Could you check a few things on this model? Use its own coordinates, in mm. Coordinates: 2 decimals unless noted, no trailing zeros. Use a Markdown table: item, result. Add a question column.
1) Will these pins go through, and if not, where does the flat tip stop? pin 1 Ø6 at (x, y) = (-6.5, -4) entering from +Z; pin 2 Ø1 at (x, z) = (-10, 6.5) entering from -Y; pin 3 Ø5 at (x, z) = (14.5, 5.5) entering from +Y; pin 4 Ø3 at (y, z) = (3.5, 1) entering from -X.
2) If we section it at A-A (y = 12.5): Give the number of separate pieces and of enclosed holes in the cut face, plus the area to 3 significant figures.
3) If I drill on L1, parallel to Y at x = -11, z = 4.5; L2, parallel to X at y = -10.5, z = 4.25; L3, parallel to Y at x = -11, z = 1.5, over which ranges is the centre line in solid material (lowest first)? Write a range as [from, to].
```python
from build123d import *

# Parameters (mm, degrees)
BASE_EXTRUDE_DEPTH      = 0.001
BASE_EXTRUDE_DEPTH_BACK = 0.001
SKETCH6_W               = 6.42
SKETCH6_H               = 6.76
SKETCH8_R               = 20.30887065
SKETCH8_R_2             = 13.5
BOSS_EXTRUDE1_DEPTH     = 6.46
CUT_EXTRUDE1_DEPTH      = 31.552378082
CUT_EXTRUDE1_DEPTH_BACK = 31.552378082


with BuildPart() as part:
    # Sketch6 → Base-Extrude (new, two sides: drawn at the far end of the back side and taken through both)
    with BuildSketch(Plane(origin=(-9.545941546, 9.545941546, 7.14), x_dir=(0.05931115895295759, 0.059311158952956106, -0.996475977054798), z_dir=(0.7046149206649441, 0.7046149206649323, 0.08387864539133799)).offset(-BASE_EXTRUDE_DEPTH_BACK)):
        with Locations((3.23, 3.4)):
            Rectangle(SKETCH6_W, SKETCH6_H)
    extrude(amount=BASE_EXTRUDE_DEPTH + BASE_EXTRUDE_DEPTH_BACK)

    # Sketch8 → Boss-Extrude1 (add)
    with BuildSketch(Plane(origin=(-0.420803093, -0.420803093, 7.069836103), x_dir=(0.9982394983905275, -0.0038244762114057976, 0.05918848903914046), z_dir=(-0.05931115895295754, -0.05931115895295616, 0.996475977054798))):
        with Locations(Location((0, 0, 0), (0, 0, 0.219513325))):
            Circle(SKETCH8_R)
        with Locations(Location((0, 0, 0), (0, 0, 0.219513325))):
            Circle(SKETCH8_R_2, mode=Mode.SUBTRACT)
    extrude(amount=-BOSS_EXTRUDE1_DEPTH)

    # Sketch9 → Cut-Extrude1 (cut, two sides: drawn at the far end of the back side and taken through both)
    with BuildSketch(Plane.XY.offset(-CUT_EXTRUDE1_DEPTH_BACK)):
        Polygon((-34.048869909, 36.453032965), (0.95291576, 1.451247296), (-1.451247296, -0.95291576), (-38.857196021, 36.453032965), align=None)
    extrude(amount=CUT_EXTRUDE1_DEPTH + CUT_EXTRUDE1_DEPTH_BACK, mode=Mode.SUBTRACT)


solid = part.part
```
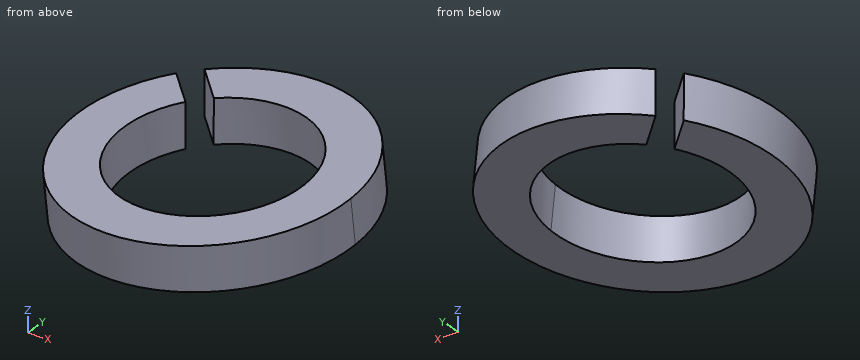
Answer sheet:
| question | item | result |
|---|---|---|
| 1 | pin 1 | through |
| 1 | pin 2 | y = 11.9 |
| 1 | pin 3 | y = 15.92 |
| 1 | pin 4 | x = -20.31 |
| 2 | separate pieces | 3 |
| 2 | enclosed holes | 0 |
| 2 | area | 116 mm2 |
| 3 | L1 | [-17.59, -8.53], [7.92, 8.6], [13.4, 16.98] |
| 3 | L2 | [-17.86, -9.11], [8.54, 17.29] |
| 3 | L3 | [-17.3, -8.12], [7.86, 8.6], [13.4, 17.04] |
